Model file for the job. Use its own axes, mm. A direction names the side the tool comes from. Coordinates: 2 decimals unless noted, no trailing zeros. Loops run counter-clockwise (first coordinate to the right, second up) from the corner with the lowest first, then second, coordinate; pieces in that order, holes last.
from build123d import *
from build123d.topology import SkipClean

# Parameters (mm, degrees)
BRACKET_BODY_DEPTH      = 30
BRACKET_BODY_SKETCH_W   = 75
BRACKET_BODY_SKETCH_H   = 15
BRACKET_BODY_2_DEPTH    = 30
COLUMN_BORE_SKETCH_R    = 20
COLUMN_BORE_40_DEPTH    = 60
COLUMN_BOSS_SKETCH_R    = 30
COLUMN_BOSS_SKETCH_R_2  = 20
COLUMN_BOSS_60_DEPTH    = 60
BASE_COLLAR_SKETCH_R    = 23
BASE_COLLAR_46_DEPTH    = 15
BODY_TRIM_CUT_SKETCH_R  = 10
BODY_TRIM_CUT_DEPTH     = 112.933015683
SIDE_BLOCK_CUT_SKETCH_R = 8
SIDE_BLOCK_CUT_DEPTH    = 158.952524513
PAD_BOSS_18MM_DEPTH     = 18
SUPPORT_RIB_DEPTH       = 5


with BuildPart() as part:
    # Bracket Body Sketch → Bracket Body (new, symmetric)
    with BuildSketch(Plane.XY):
        Polygon((-60, 15), (-60, 60), (-45, 60), (-45, 30), (0, 30), (0, 15), align=None)
    extrude(amount=BRACKET_BODY_DEPTH, both=True)


with BuildPart() as body_2:
    # Bracket Body Sketch → Bracket Body 2 (new, symmetric)
    with BuildSketch(Plane.XY):
        with Locations((37.5, 7.5)):
            Rectangle(BRACKET_BODY_SKETCH_W, BRACKET_BODY_SKETCH_H)
    extrude(amount=BRACKET_BODY_2_DEPTH, both=True)


with BuildPart() as column_bore_40_tool:
    # Column Bore Sketch → Column Bore _40 (new body)
    with BuildSketch(Plane(origin=(0, 0, 0), x_dir=(1, 0, 0), z_dir=(0, 1, 0))):
        Circle(COLUMN_BORE_SKETCH_R)
    extrude(amount=COLUMN_BORE_40_DEPTH)


with BuildPart() as part_1:
    add(part.part)

    # Column Bore _40: cut by column_bore_40_tool
    add(column_bore_40_tool.part, mode=Mode.SUBTRACT)



with BuildPart() as body_2_1:
    add(body_2.part)

    # Column Bore _40: cut by column_bore_40_tool
    add(column_bore_40_tool.part, mode=Mode.SUBTRACT)


with BuildPart() as part_2:
    add(part_1.part)

    add(body_2_1.part)  # Column Boss _60 merges body 2
    # Column Boss Sketch → Column Boss _60 (add)
    with BuildSketch(Plane(origin=(0, 0, 0), x_dir=(1, 0, 0), z_dir=(0, 1, 0))):
        with Locations(Location((0, 0, 0), (0, 0, 270))):
            Circle(COLUMN_BOSS_SKETCH_R)
        with Locations(Location((0, 0, 0), (0, 0, 270))):
            Circle(COLUMN_BOSS_SKETCH_R_2, mode=Mode.SUBTRACT)
    extrude(amount=COLUMN_BOSS_60_DEPTH)

    # Base Collar Sketch → Base Collar _46 (add)
    with BuildSketch(Plane(origin=(0, 0, 0), x_dir=(1, 0, 0), z_dir=(0, 1, 0))):
        with Locations((75, 0)):
            Circle(BASE_COLLAR_SKETCH_R)
    extrude(amount=BASE_COLLAR_46_DEPTH)

    # Body Trim Cut Sketch → Body Trim Cut (cut, through all)
    with SkipClean():  # the faces are left unmerged after this step: merging them gives an invalid solid
        with BuildSketch(Plane(origin=(0, 15, 0), x_dir=(1, 0, 0), z_dir=(0, 1, 0))):
            with Locations(Location((75, 0, 0), (0, 0, 270))):
                Circle(BODY_TRIM_CUT_SKETCH_R)
            with BuildLine():
                Line((75, 23), (19.261360284, 23))
                ThreePointArc((19.261360284, 23), (10.246950766, 28.19574436), (0, 30))
                Line((0, 30), (75, 30))
                Line((75, 30), (75, 23))
            make_face()
            with BuildLine():
                Line((75, -23), (75, -30))
                Line((75, -30), (0, -30))
                ThreePointArc((0, -30), (10.246950766, -28.19574436), (19.261360284, -23))
                Line((19.261360284, -23), (75, -23))
            make_face()
        extrude(amount=-BODY_TRIM_CUT_DEPTH, mode=Mode.SUBTRACT)

    # Side Block Cut Sketch → Side Block Cut (cut, through all)
    with SkipClean():  # the faces are left unmerged after this step: merging them gives an invalid solid
        with BuildSketch(Plane(origin=(-45, 0, 0), x_dir=(0, 0, -1), z_dir=(1, 0, 0))):
            with Locations(Location((-17.5, 45, 0), (0, 0, 90))):
                Circle(SIDE_BLOCK_CUT_SKETCH_R)
            with Locations(Location((17.5, 45, 0), (0, 0, 270))):
                Circle(SIDE_BLOCK_CUT_SKETCH_R)
        extrude(amount=-SIDE_BLOCK_CUT_DEPTH, mode=Mode.SUBTRACT)

    # Pad Boss Sketch → Pad Boss 18mm (add)
    with SkipClean():  # the faces are left unmerged after this step: merging them gives an invalid solid
        with BuildSketch(Plane(origin=(-45, 0, 0), x_dir=(0, 0, -1), z_dir=(1, 0, 0))):
            Polygon((0, 60), (5, 60), (5, 30), (-5, 30), (-5, 60), align=None)
        extrude(amount=PAD_BOSS_18MM_DEPTH)

    # Support Rib Sketch → Support Rib (add, symmetric)
    with BuildSketch(Plane.XY):
        Polygon((30, 15), (55, 15), (30, 60), (20, 60), (20, 15), align=None)
    extrude(amount=SUPPORT_RIB_DEPTH, both=True)


solid = part_2.part
Q1. Slice it at A-A (y = 44). List the corners of the cut face in (x, z), and give its area (3 significant figures).
Answers:
outline: (-60, -30) - (-45, -30) - (-45, -25.44) - (-60, -25.44) - close; (-60, -9.56) - (-45, -9.56) - (-45, -5) - (-29.58, -5) arc R30 ccw to (29.58, -5) - (38.89, -5) - (38.89, 5) - (29.58, 5) arc R30 ccw to (-29.58, 5) - (-45, 5) - (-45, 9.56) - (-60, 9.56) - close; (-60, 25.44) - (-45, 25.44) - (-45, 30) - (-60, 30) - close; hole circle Ø40 at (0, 0)
area: 2,240 mm2
Q2. Mould opens along Y. For faces 6 (the flat face through (58, 15, 0)), 7 (the cylindrical face through (-52.395, 51.349, -12.632)), 8 (the flat face through (-37, 45, -5)) say: +Y half, -Y half, draft (parallel to the pull), parting line (faces both ways), or undercut.
Answers:
face 6: +Y half
face 7: undercut
face 8: draft
Q3. Slice it at C-C (x = -37). List the corners of the cut face in (y, z), and give its area (3 significant figures).
Answers:
outline: (15, -30) - (30, -30) - (30, -5) - (60, -5) - (60, 5) - (30, 5) - (30, 30) - (15, 30) - close
area: 1,200 mm2
Q4. Slice it at D-D (y = 27.5). List the corners of the cut face in (x, z), and give its area (3 significant figures).
Answers:
outline: (-60, -30) - (0, -30) arc R30 ccw to (29.58, -5) - (48.06, -5) - (48.06, 5) - (29.58, 5) arc R30 ccw to (0, 30) - (-60, 30) - close; hole circle Ø40 at (0, 0)
area: 3,940 mm2
Q5. Which spindle directions (+Z, -Z, +X, -X, +Y, -Y) get a long thin tool onto all of the face, cutting with end or side? Do faces 1 (the flat face through (39, 33, -5)), 2 (the flat face through (39, 33, 5)), 3 (the flat face through (-36, 28, -30)), 4 (the flat face through (-43, 15, 0)), 5 (the flat face through (-33, 30, 20)). Say none if no direction does.
Answers:
face 1: -Z, +X, +Y
face 2: +Z, +X, +Y
face 3: -Z, +X, -X, +Y, -Y
face 4: -X, -Y
face 5: +Z, +Y
Q6. Drill centre lines: line 1 (X direction, y = 10.5, z = 0.5); line 2 (X direction, y = 54, z = 5.5); line 3 (Z direction, x = 0, y = 41). Where is each one in solid material? Low to high.
Answers:
line 1: x = -30 to -19.99, 19.99 to 65.01, 84.99 to 97.99
line 2: x = -60 to -45, -29.49 to -19.23, 19.23 to 29.49
line 3: z = -30 to -20, 20 to 30
Q7. Flat gauge pins, fed straight in: P1, Ø18, axis at x = 75, z = 0, coming from the -Y side; P2, Ø7.5, axis at y = 38, z = 13.5, coming from the +X side; P3, Ø4, axis at x = 37.5, z = 11, coming from the +Y side; P4, Ø20.5, axis at x = 48.5, y = 43.5, coming from the +Z side. Where does each tip first touch, or does it go through?
Answers:
P1: passes through
P2: stops at x = 28.37
P3: stops at y = 15
P4: stops at z = 5
Q8. Slice it at B-B (z = 0). List the corners of the cut face in (x, y), and give its area (3 significant figures).
Answers:
outline: (-60, 15) - (-30, 15) - (-30, 0) - (-20, 0) - (-20, 60) - (-60, 60) - close; (20, 0) - (65, 0) - (65, 15) - (55, 15) - (30, 60) - (20, 60) - close; (85, 0) - (98, 0) - (98, 15) - (85, 15) - close
area: 3,830 mm2
